from build123d import *

# Parameters (mm, degrees)
EXTRUDE_1_DEPTH = 170


with BuildPart() as part:
    # 草图1 → 凸台-拉伸1 (new body)
    with BuildSketch(Plane.XY):
        with BuildLine():
            Line((0, 75), (-1610, 75))
            ThreePointArc((-1610, 75), (-1685, 0), (-1610, -75))
            Line((-1610, -75), (0, -75))
            ThreePointArc((0, -75), (75, 0), (0, 75))
        make_face()
        with BuildLine():
            Line((0, 60), (-1610, 60))
            ThreePointArc((-1610, 60), (-1670, 0), (-1610, -60))
            Line((-1610, -60), (0, -60))
            ThreePointArc((0, -60), (60, 0), (0, 60))
        make_face(mode=Mode.SUBTRACT)
    extrude(amount=EXTRUDE_1_DEPTH)


solid = part.part
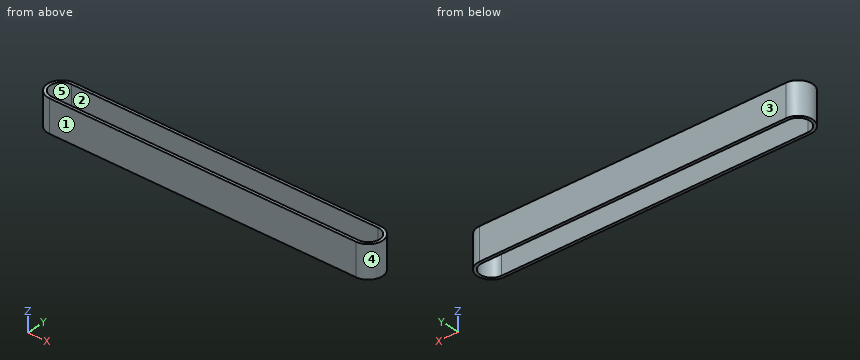
Could you check a few things on this model? Use its own coordinates, in mm. Face numbers are marked on the shaded views. A direction names the side the tool comes from. Round coordinates to 2 decimals unless told otherwise and drop trailing zeros. Loops run counter-clockwise (first coordinate to the right, second up) from the corner with the lowest first, then second, coordinate; pieces in that order, holes last. Notation, with made-up numbers: (46.25, -39.5) - (61.25, -39.5) arc R27 ccw to (61.25, -23.5) - close; hole circle Ø10 at (40, -33). An arc over 180 degrees is marked (long way). Write item = value, one per line.
1) I'm going to push flat-ended pins straight in: P1, Ø3, axis at y = -30, z = 83.5, coming from the +X side; P2, Ø1.5, axis at y = 2, z = 31.5, coming from the -X side; P3, Ø2, axis at y = -26.5, z = 21.5, coming from the +X side. Where does each tip first touch, or does it pass through?
Computed:
P1 = 69.37
P2 = -1684.99
P3 = 70.53
2) On a 3-axis mill with a long thin cutter (end or side, diameter ignored), from which of +Z, -Z, +X, -X, +Y, -Y can I reach the whole of each face in a straight line? I mean the marked faces 1 and 2. Say none if no direction works.
Computed:
face_1 = +Z, -Z, +X, -X, -Y
face_2 = +Z, -Z
3) If we mould it in two halves opening along X, with no side actions, what happens to the marked faces 3, 4 and 5? For each: pulls with the +X half, pulls with the -X half, needs draft (parallel to the pull), parting line crosses it, or undercut.
Computed:
face_3 = needs draft
face_4 = pulls with the +X half
face_5 = undercut
4) Imagine slicing it at C-C (z = 124). Please give me the cut outline in (x, y).
Computed:
outline = (-1610, -75) - (0, -75) arc R75 ccw to (0, 75) - (-1610, 75) arc R75 ccw to start; hole (-1610, -60) - (0, -60) arc R60 ccw to (0, 60) - (-1610, 60) arc R60 ccw to start
5) I need wall thicknesses on line 1 along Y through (x, z) = (-1259, 139); line 2 along Y through (x, z) = (2.5, 30); line 3 along X through (y, z) = (21.5, 20.5). Which ranges of each line are inside material? Lowest first, please. Write a range as from..to.
Computed:
line_1 = -75..-60, 60..75
line_2 = -74.96..-59.95, 59.95..74.96
line_3 = -1681.85..-1666.02, 56.02..71.85
6) Imagine slicing it at A-A (y = 0). Please give me the cut outline in (x, z), and give its area (3 significant figures).
Computed:
outline = (-1685, 0) - (-1670, 0) - (-1670, 170) - (-1685, 170) - close; (60, 0) - (75, 0) - (75, 170) - (60, 170) - close
area = 5,100 mm2
7) Imagine slicing it at B-B (x = -909). Please give me the cut outline in (y, z), and give its area (3 significant figures).
Computed:
outline = (-75, 0) - (-60, 0) - (-60, 170) - (-75, 170) - close; (60, 0) - (75, 0) - (75, 170) - (60, 170) - close
area = 5,100 mm2
